For this review, use the dimensioned drawing (mm, ordinates from the lowest corner) and the shaded views. Give positions to 0.01 mm unless a question says otherwise; leave off trailing zeros. Write each loop counter-clockwise with the first axis right and the second up, starting at its lowest first coordinate (ties: lowest second). Pieces come first, ordered by that corner, then holes.
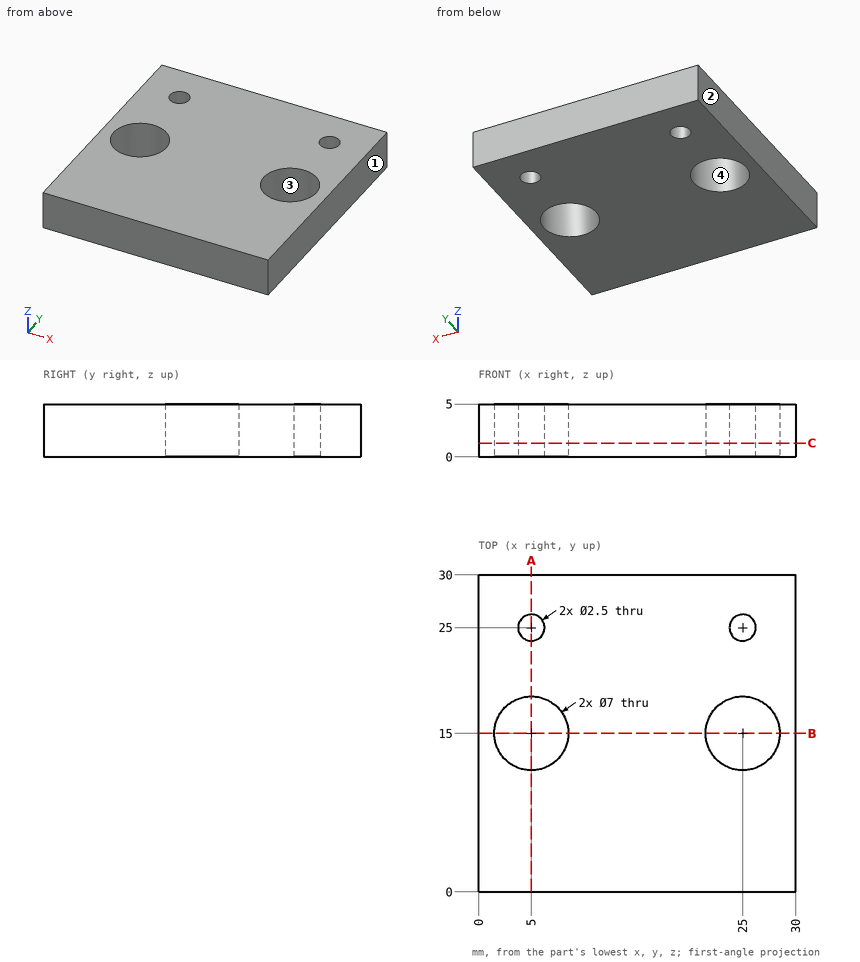
(1) We need section A-A (x = 5). Write out the cut boundary in (y, z).
(2) The part is to be moulded in two halves that separate along X. For the marked faces 1, 2, 3 and 4, say which applies: +X half, -X half, draft (parallel to the pull), parting line (faces both ways), or undercut.
(3) For L1, parallel to X at y = 25, z = 1.4; L2, parallel to Y at x = 25, z = 1.15; L3, parallel to X at y = 12.75, z = 0.55, list the stretches that pass through material, from the lowest coordinate up.
(4) We need section B-B (y = 15). Write out the cut boundary in (x, z).
(5) We need section C-C (z = 1.3). Write out the cut boundary in (x, y), and give its area (3 significant figures).
(6) Clearance check with a flat-ended pin moving along its axis: pin 1 Ø8 at (x, y) = (18.5, 26.5) entering from -Z. State where the tip first meets the part, or that it passes through.
The answers:
1. outline: (0, 0) - (11.5, 0) - (11.5, 5) - (0, 5) - close; (18.5, 0) - (23.75, 0) - (23.75, 5) - (18.5, 5) - close; (26.25, 0) - (30, 0) - (30, 5) - (26.25, 5) - close
2. face 1: +X half
2. face 2: -X half
2. face 3: undercut
2. face 4: undercut
3. L1: x = 0 to 3.75, 6.25 to 23.75, 26.25 to 30
3. L2: y = 0 to 11.5, 18.5 to 23.75, 26.25 to 30
3. L3: x = 0 to 2.32, 7.68 to 22.32, 27.68 to 30
4. outline: (0, 0) - (1.5, 0) - (1.5, 5) - (0, 5) - close; (8.5, 0) - (21.5, 0) - (21.5, 5) - (8.5, 5) - close; (28.5, 0) - (30, 0) - (30, 5) - (28.5, 5) - close
5. outline: (0, 0) - (30, 0) - (30, 30) - (0, 30) - close; hole circle Ø7 at (5, 15); hole circle Ø2.5 at (5, 25); hole circle Ø7 at (25, 15); hole circle Ø2.5 at (25, 25)
5. area: 813 mm2
6. pin 1: stops at z = 0
